```python
from build123d import *

# Parameters (mm, degrees)
SKETCH1_W           = 79.884759576
SKETCH1_H           = 30.264710677
BOSS_EXTRUDE1_DEPTH = 20
SKETCH2_W           = 79.884759576
SKETCH2_H           = 30.088424062
BOSS_EXTRUDE2_DEPTH = 5
SKETCH3_R           = 3.245829629
CUT_EXTRUDE1_DEPTH  = 47
FILLET1_R           = 1
SKETCH4_R           = 3.674588618
BOSS_EXTRUDE3_DEPTH = 7
SKETCH5_R           = 3.674588618
BOSS_EXTRUDE4_DEPTH = 3.5
SKETCH6_W           = 7.683150555
SKETCH6_H           = 33.560004606
SKETCH6_R           = 2
BOSS_EXTRUDE5_DEPTH = 3


with BuildPart() as part:
    # Sketch1 → Boss-Extrude1 (new, symmetric)
    with BuildSketch(Plane.XY):
        with Locations((0, 50.939731052)):
            Rectangle(SKETCH1_W, SKETCH1_H)
    extrude(amount=BOSS_EXTRUDE1_DEPTH, both=True)

    # Sketch2 → Boss-Extrude2 (add)
    with BuildSketch(Plane.XZ.offset(-35.807375713)):
        Rectangle(SKETCH2_W, SKETCH2_H)
    extrude(amount=BOSS_EXTRUDE2_DEPTH)

    # Sketch3 → Cut-Extrude1 (cut)
    with BuildSketch(Plane(origin=(0, 66.07208639, 0), x_dir=(1, 0, 0), z_dir=(0, 1, 0))):
        with Locations((-21.223926361, 20)):
            Circle(SKETCH3_R)
        with Locations((21.223926361, 20)):
            Circle(SKETCH3_R)
        with Locations((21.223926361, -20)):
            Circle(SKETCH3_R)
        with Locations((-21.223926361, -20)):
            Circle(SKETCH3_R)
    extrude(amount=-CUT_EXTRUDE1_DEPTH, mode=Mode.SUBTRACT)

    # Fillet1
    fillet1_edges = [part.edges().sort_by_distance(p)[0] for p in [
        (-39.942379788, 50.939731051, 20),
        (39.942379788, 50.939731051, 20),
        (-39.942379788, 50.939731051, -20),
        (39.942379788, 50.939731051, -20),
    ]]
    fillet(fillet1_edges, radius=FILLET1_R)

    # Sketch4 → Boss-Extrude3 (add)
    with BuildSketch(Plane.XY.offset(13.044212031)):
        with BuildLine():
            Line((-39.942379788, 30.807375713), (-39.942379788, 29.427732571))
            ThreePointArc((-39.942379788, 29.427732571), (-39.780068199, 28.164098588), (-39.303671451, 26.98250558))
            Line((-39.303671451, 26.98250558), (-31.815081757, 13.625903547))
            ThreePointArc((-31.815081757, 13.625903547), (-25.689559132, 11.020522164), (-21.620670757, 16.288746435))
            Line((-21.620670757, 16.288746435), (-21.620670757, 30.807375713))
            Line((-21.620670757, 30.807375713), (-39.942379788, 30.807375713))
        make_face()
        with Locations((-27.065651732, 16.288746435)):
            Circle(SKETCH4_R, mode=Mode.SUBTRACT)
    boss_extrude3 = extrude(amount=-BOSS_EXTRUDE3_DEPTH)

    # Mirror1: Boss-Extrude3 across plane
    add(boss_extrude3.mirror(Plane.XY))

    # Sketch5 → Boss-Extrude4 (add, symmetric)
    with BuildSketch(Plane.XY):
        with BuildLine():
            Line((21.620670757, 16.288746435), (21.620670757, 30.807375713))
            Line((21.620670757, 30.807375713), (39.942379788, 30.807375713))
            Line((39.942379788, 30.807375713), (39.942379788, 29.427732571))
            ThreePointArc((39.942379788, 29.427732571), (39.780068199, 28.164098588), (39.303671451, 26.98250558))
            Line((39.303671451, 26.98250558), (31.815081757, 13.625903547))
            ThreePointArc((31.815081757, 13.625903547), (25.689559132, 11.020522164), (21.620670757, 16.288746435))
        make_face()
        with Locations((27.065651732, 16.288746435)):
            Circle(SKETCH5_R, mode=Mode.SUBTRACT)
    extrude(amount=BOSS_EXTRUDE4_DEPTH, both=True)

    # Sketch6 → Boss-Extrude5 (add)
    # profile 1 of 2: a face of its own
    with BuildSketch(Plane(origin=(0, 66.07208639, 0), x_dir=(1, 0, 0), z_dir=(0, 1, 0))):
        with Locations((-43.783955066, 0)):
            Rectangle(SKETCH6_W, SKETCH6_H)
        with Locations(Location((-43.783955066, 9.635125017, 0), (0, 0, 270))):
            Circle(SKETCH6_R, mode=Mode.SUBTRACT)
        with Locations(Location((-43.783955066, -9.635125017, 0), (0, 0, 90))):
            Circle(SKETCH6_R, mode=Mode.SUBTRACT)
    # profile 2 of 2: a face of its own
    with BuildSketch(Plane(origin=(0, 66.07208639, 0), x_dir=(1, 0, 0), z_dir=(0, 1, 0))):
        with Locations((43.783955066, 0)):
            Rectangle(SKETCH6_W, SKETCH6_H)
        with Locations(Location((43.783955066, -9.635125017, 0), (0, 0, 270))):
            Circle(SKETCH6_R, mode=Mode.SUBTRACT)
        with Locations(Location((43.783955066, 9.635125017, 0), (0, 0, 90))):
            Circle(SKETCH6_R, mode=Mode.SUBTRACT)
    extrude(amount=-BOSS_EXTRUDE5_DEPTH)


solid = part.part
```
Build history of the part. All positions in model axes, mm. A direction names the side the tool comes from. Give positions to 0.01 mm unless a question says otherwise; leave off trailing zeros. Loops run counter-clockwise (first coordinate to the right, second up) from the corner with the lowest first, then second, coordinate; pieces in that order, holes last. Notation, with made-up numbers: (62, 15.5) -> (99, 15.5) arc R31 ccw to (99, 39.5) -> close; hole circle Ø4 at (89.25, 65). An arc over 180 degrees is marked (long way). One line per question, with ' | ' between items. Start each with the question number.
1) Pin check, flat tips, straight feed: pin 1 (0.9 mm diameter, centred on x = 45, y = 64.5, fed in from -Z); pin 2 (1.5 mm diameter, centred on y = 18.5, z = 8.5, fed in from +X); pin 3 (5.5 mm diameter, centred on x = -30.5, y = 18.5, fed in from +Z). Stop position of each tip, or through.
2) Probe L1, parallel to X at y = 54, z = -17.5; L2, parallel to Y at x = 39, z = -10; L3, parallel to Y at x = 23.5, z = 16.5. List the from-to ranges inside material, lowest first.
3) Cut at A-A (z = 0.5). Give the cut face in (x, y), plus the area to 3 significant figures.
4) Two-plate mould, pull along X, no slides. Class faces 4 (the cylindrical face through (21.153, 51.152, -16.755)), 5 (the flat face through (32, 51, 20)), 6 (the flat face through (-21.621, 23, 10)): released by +X, released by -X, zero draft, split by the parting line, or undercut.
5) Cut at B-B (x = 11). Give the cut face in (y, z), plus the area to 3 significant figures.
6) Cut at D-D (x = 29). Give the cut face in (y, z), plus the area to 3 significant figures.
7) Cut at C-C (z = 10.5). Give the cut face in (x, y), plus the area to 3 significant figures.
8) 3-axis set-ups, long thin cutter, end or side, ignore diameter. For faces 1 (the flat face through (-1, 35.807, 18)), 2 (the flat face through (-1, 33, -15.044)), 3 (the flat face through (-29, 23, -6.044)): which of +Z, -Z, +X, -X, +Y, -Y reach the whole face in a straight line?
Return value:
1) pin 1: z = -16.78 | pin 2: x = -21.62 | pin 3: z = 13.04
2) L1: -39.94 to -23.29, -19.15 to 19.15, 23.29 to 39.94 | L2: 30.81 to 66.07 | L3: 35.81 to 66.07
3) outline: (-47.63, 63.07) -> (-39.94, 63.07) -> (-39.94, 30.81) -> (21.62, 30.81) -> (21.62, 16.29) arc R5.44 ccw to (31.82, 13.63) -> (39.3, 26.98) arc R5 ccw to (39.94, 29.43) -> (39.94, 63.07) -> (47.63, 63.07) -> (47.63, 66.07) -> (-47.63, 66.07) -> close; hole circle Ø7.35 at (27.07, 16.29) | area: 3,090 mm^2
4) face 4: undercut | face 5: zero draft | face 6: released by +X
5) outline: (30.81, -15.04) -> (35.81, -15.04) -> (35.81, -20) -> (66.07, -20) -> (66.07, 20) -> (35.81, 20) -> (35.81, 15.04) -> (30.81, 15.04) -> close | area: 1,360 mm^2
6) outline: (11.2, -3.5) -> (13.16, -3.5) -> (13.16, 3.5) -> (11.2, 3.5) -> close; (19.41, -3.5) -> (30.81, -3.5) -> (30.81, -15.04) -> (35.81, -15.04) -> (35.81, -20) -> (66.07, -20) -> (66.07, 20) -> (35.81, 20) -> (35.81, 15.04) -> (30.81, 15.04) -> (30.81, 3.5) -> (19.41, 3.5) -> close | area: 1,450 mm^2
7) outline: (-47.63, 63.07) -> (-45.59, 63.07) -> (-45.59, 66.07) -> (-47.63, 66.07) -> close; (-41.98, 63.07) -> (-39.94, 63.07) -> (-39.94, 29.43) arc R5 ccw to (-39.3, 26.98) -> (-31.82, 13.63) arc R5.44 ccw to (-21.62, 16.29) -> (-21.62, 30.81) -> (39.94, 30.81) -> (39.94, 63.07) -> (41.98, 63.07) -> (41.98, 66.07) -> (-41.98, 66.07) -> close; (45.59, 63.07) -> (47.63, 63.07) -> (47.63, 66.07) -> (45.59, 66.07) -> close; hole circle Ø7.35 at (-27.07, 16.29) | area: 3,070 mm^2
8) face 1: +Z, +X, -X, -Y | face 2: -Z, +X, -X, -Y | face 3: +X, -X, -Y
